from build123d import *

# Parameters (mm, degrees)
EXTRUDE_1_DEPTH     = 550
CUT_EXTRUDE_1_DEPTH = 578.711000415


with BuildPart() as part:
    # 草图1 → 凸台-拉伸1 (new, symmetric)
    with BuildSketch(Plane.XY):
        Polygon((0, 125), (10, 125), (10, 10), (125, 10), (125, 0), (0, 0), align=None)
    extrude(amount=EXTRUDE_1_DEPTH, both=True)

    # 草图2 → 切除-拉伸1 (cut, through all)
    with BuildSketch(Plane(origin=(125, 0, 0), x_dir=(0, 0, -1), z_dir=(1, 0, 0))):
        Polygon((-550, 0), (-550, 125), (-425, 125), align=None)
        Polygon((425, 125), (550, 0), (550, 125), align=None)
    extrude(amount=-CUT_EXTRUDE_1_DEPTH, mode=Mode.SUBTRACT)


solid = part.part
Could you check a few things on this model? Use its own coordinates, in mm. A direction names the side the tool comes from. Coordinates: 2 decimals unless noted, no trailing zeros. Loops run counter-clockwise (first coordinate to the right, second up) from the corner with the lowest first, then second, coordinate; pieces in that order, holes last.
1. Imagine slicing it at B-B (y = 89.5). Please give me the cut outline in (x, z), and give its area (3 significant figures).
2. For faces 1 (the face through (7, 35, 515)), 2 (the face through (10, 68, 8)), which set-ups out of +Z, -Z, +X, -X, +Y, -Y let a thin tool reach every point of the face, with its end or its side?
3. Imagine slicing it at C-C (x = 73). Please give me the cut outline in (y, z).
4. I need wall thicknesses on L1, parallel to X at y = 20, z = -416.5; L2, parallel to Z at x = 8.5, y = 71.5. Which ranges of each line are inside material? Lowest first, please.
5. Imagine slicing it at D-D (z = -460). Please give me the cut outline in (x, y).
6. For P1, Ø2, axis at y = 57, z = -281.5, coming from the +X side; P2, Ø5, axis at x = 90, z = 230, coming from the +Y side, each with a flat end and sliding along its axis, tell me the tip position at first contact or that it passes through.
7. Imagine slicing it at A-A (z = 434.5). Please give me the cut outline in (x, y).
Computed values:
1. outline: (0, -460.5) - (10, -460.5) - (10, 460.5) - (0, 460.5) - close
1. area: 9,210 mm2
2. face 1: +Z, +X, -X, +Y
2. face 2: +Z, -Z, +X, +Y
3. outline: (0, -550) - (10, -540) - (10, 540) - (0, 550) - close
4. L1: x = 0 to 10
4. L2: z = -478.5 to 478.5
5. outline: (0, 0) - (125, 0) - (125, 10) - (10, 10) - (10, 90) - (0, 90) - close
6. P1: stops at x = 10
6. P2: stops at y = 10
7. outline: (0, 0) - (125, 0) - (125, 10) - (10, 10) - (10, 115.5) - (0, 115.5) - close
